Build history of the part. All positions in model axes, mm. A direction names the side the tool comes from. Round coordinates to 2 decimals unless told otherwise and drop trailing zeros. Write each loop counter-clockwise with the first axis right and the second up, starting at its lowest first coordinate (ties: lowest second). Pieces come first, ordered by that corner, then holes.
Item 1: Band-saw the part on D-D, the plane y = 41.5. Write the cut outline in (x, z), then the cut area to 3 significant figures.
Item 2: Wall check: probe 1 along X at (y, z) = (57, 62); probe 2 along Y at (x, z) = (11.5, 108); probe 3 along Y at (x, z) = (11.5, 71.5). Give the ranges that are in metal, low to high.
Item 3: 3-axis set-ups, long thin cutter, end or side, ignore diameter. For faces 1 (the flat face through (41, 35, 25)), 2 (the cylindrical face through (69.41, 64.44, 39.44)), 3 (the conical face through (24.565, 48.562, 9.601)): which of +Z, -Z, +X, -X, +Y, -Y reach the whole face in a straight line?
Item 4: Band-saw the part on A-A, the plane y = 12.5. Write the cut outline in (x, z).
Item 5: Band-saw the part on C-C, the plane z = 28. Write the cut outline in (x, y).
Item 6: Mould opens along Z. For faces 4 (the flat face through (80, 42, 72)), 5 (the flat face through (7, 56, 80)), 6 (the cylindrical face through (45.753, 51.494, 101.912)) say: +Z half, -Z half, draft (parallel to the pull), parting line (faces both ways), or undercut.
Item 7: Drop flat-ended pins along their axis: pin 1 Ø12.5 at (x, y) = (68.5, 12.5) entering from -Z; pin 2 Ø11 at (x, y) = (68.5, 57.5) entering from +Z; pin 3 Ø14.5 at (x, y) = (11.5, 12.5) entering from -Z; pin 4 Ø8 at (x, z) = (55, 10) entering from -Y. Give the stop position or say it passes through.
Item 8: Band-saw the part on B-B, the plane x = 66.5. Write the cut outline in (y, z), then the cut area to 3 significant figures.
```python
from build123d import *

# Parameters (mm, degrees)
SKETCH_1_W             = 80
SKETCH_1_H             = 70
EXTRUDE_1_DEPTH        = 118.5
SKETCH_4_R             = 7
CUT_EXTRUDE_1_DEPTH    = 80
SKETCH_5_R             = 4.5
CUT_EXTRUDE_2_DEPTH    = 160.192493542
SKETCH_6_W             = 80
SKETCH_6_H             = 35
CUT_EXTRUDE_3_DEPTH    = 50
M16X1_5_1_D            = 14.5
M16X1_5_1_DEPTH        = 36.5
M16X1_5_1_TIP          = 4.356239488
HOLE_WIZARD_M8_1_D     = 6.8
HOLE_WIZARD_M8_1_DEPTH = 19.75
HOLE_WIZARD_M8_1_TIP   = 2.042926105
CHAMFER_1_SIZE         = 2


with BuildPart() as part:
    # 草图1 → 凸台-拉伸1 (new body)
    with BuildSketch(Plane.XY):
        with Locations((40, 35)):
            Rectangle(SKETCH_1_W, SKETCH_1_H)
    extrude(amount=EXTRUDE_1_DEPTH)

    # 草图4 → 切除-拉伸1 (cut)
    with BuildSketch(Plane(origin=(0, 0, 0), x_dir=(-1, 0, 0), z_dir=(0, 0, -1))):
        with Locations((-11.5, 57.5)):
            Circle(SKETCH_4_R)
        with Locations((-11.5, 12.5)):
            Circle(SKETCH_4_R)
        with Locations((-68.5, 57.5)):
            Circle(SKETCH_4_R)
        with Locations((-68.5, 12.5)):
            Circle(SKETCH_4_R)
    extrude(amount=-CUT_EXTRUDE_1_DEPTH, mode=Mode.SUBTRACT)

    # 草图5 → 切除-拉伸2 (cut, through all)
    with BuildSketch(Plane(origin=(0, 0, 0), x_dir=(-1, 0, 0), z_dir=(0, 0, -1))):
        with Locations((-68.5, 57.5)):
            Circle(SKETCH_5_R)
        with Locations((-11.5, 57.5)):
            Circle(SKETCH_5_R)
        with Locations((-11.5, 12.5)):
            Circle(SKETCH_5_R)
        with Locations((-68.5, 12.5)):
            Circle(SKETCH_5_R)
    extrude(amount=-CUT_EXTRUDE_2_DEPTH, mode=Mode.SUBTRACT)

    # 草图6 → 切除-拉伸3 (cut)
    with BuildSketch(Plane(origin=(0, 0, 0), x_dir=(-1, 0, 0), z_dir=(0, 0, -1))):
        with Locations((-40, 17.5)):
            Rectangle(SKETCH_6_W, SKETCH_6_H)
    extrude(amount=-CUT_EXTRUDE_3_DEPTH, mode=Mode.SUBTRACT)

    # M16x1.5 螺纹孔1
    with Locations(Plane(origin=(0, 70, 0), x_dir=(1, 0, 0), z_dir=(0, 1, 0))):
        with Locations((40, -97.5)):
            Hole(M16X1_5_1_D / 2, depth=M16X1_5_1_DEPTH)
            with Locations((0, 0, -(M16X1_5_1_DEPTH + M16X1_5_1_TIP / 2))):  # 118° drill point
                Cone(0, M16X1_5_1_D / 2, M16X1_5_1_TIP, mode=Mode.SUBTRACT)

    # M8 螺纹孔1
    with Locations(Plane(origin=(0, 70, 0), x_dir=(1, 0, 0), z_dir=(0, 1, 0))):
        with Locations((55, -10), (25, -10)):
            Hole(HOLE_WIZARD_M8_1_D / 2, depth=HOLE_WIZARD_M8_1_DEPTH)
            with Locations((0, 0, -(HOLE_WIZARD_M8_1_DEPTH + HOLE_WIZARD_M8_1_TIP / 2))):  # 118° drill point
                Cone(0, HOLE_WIZARD_M8_1_D / 2, HOLE_WIZARD_M8_1_TIP, mode=Mode.SUBTRACT)

    # 倒角1
    chamfer_1_edges = [part.edges().sort_by_distance(p)[0] for p in [
        (80, 35, 25),
        (0, 35, 25),
        (0, 70, 59.25),
        (80, 70, 59.25),
        (80, 0, 84.25),
        (0, 0, 84.25),
    ]]
    chamfer(chamfer_1_edges, length=CHAMFER_1_SIZE)


solid = part.part
```
Results:
1. outline: (0, 0) - (80, 0) - (80, 118.5) - (0, 118.5) - close; hole circle Ø14.5 at (40, 97.5)
1. area: 9,310 mm2
2. probe 1: x = 0 to 4.52, 18.48 to 61.52, 75.48 to 80
2. probe 2: y = 0 to 8, 17 to 53, 62 to 70
2. probe 3: y = 0 to 5.5, 19.5 to 50.5, 64.5 to 70
3. face 1: -Z, +X, -X, -Y
3. face 2: -Z
3. face 3: +Y
4. outline: (0, 50) - (4.5, 50) - (4.5, 80) - (7, 80) - (7, 118.5) - (0, 118.5) - close; (16, 80) - (18.5, 80) - (18.5, 50) - (61.5, 50) - (61.5, 80) - (64, 80) - (64, 118.5) - (16, 118.5) - close; (73, 80) - (75.5, 80) - (75.5, 50) - (80, 50) - (80, 118.5) - (73, 118.5) - close
5. outline: (0, 37) - (2, 35) - (78, 35) - (80, 37) - (80, 68) - (78, 70) - (2, 70) - (0, 68) - close; hole circle Ø14 at (11.5, 57.5); hole circle Ø14 at (68.5, 57.5)
6. face 4: draft
6. face 5: -Z half
6. face 6: undercut
7. pin 1: stops at z = 80
7. pin 2: stops at z = 118.5
7. pin 3: stops at z = 50
7. pin 4: stops at y = 35
8. outline: (0, 50) - (5.79, 50) - (5.79, 80) - (8.47, 80) - (8.47, 118.5) - (0, 118.5) - close; (16.53, 80) - (19.21, 80) - (19.21, 50) - (35, 50) - (35, 0) - (50.79, 0) - (50.79, 80) - (53.47, 80) - (53.47, 118.5) - (16.53, 118.5) - close; (61.53, 80) - (64.21, 80) - (64.21, 0) - (70, 0) - (70, 118.5) - (61.53, 118.5) - close
8. area: 4,450 mm2
